Geometry: final body of the model. Coordinates: model frame, mm. Face numbers are marked on the shaded views. A direction names the side the tool comes from. Coordinates: 2 decimals unless noted, no trailing zeros. Write each loop counter-clockwise with the first axis right and the second up, starting at its lowest first coordinate (ties: lowest second). Pieces come first, ordered by that corner, then holes. Notation, with made-up numbers: M 74,-21.5 L 126,-21.5 A10 ccw 126,-4.5 Z; hole C 24,20.5 d8. An arc over 180 degrees is marked long. Write item = value, one per line. Start each with the question number.
Item 1: Reachability of the marked faces 1, 2 and 3 from +Z, -Z, +X, -X, +Y, -Y: full face, straight path, thin tool, end or side. Return the list, or none.
Item 2: Ray query, L1, parallel to X at y = 2.8, z = 0; L2, parallel to X at y = 0.7, z = 0; L3, parallel to Z at x = -14.5, y = 2.5. Return the intervals inside material, ascending. Write a range as [from, to].
Item 3: Section D-D on x = 16.5. Output: boundary loops of the cut face in (y, z).
Item 4: First-contact query: pin 1 Ø10 at (x, z) = (-3.5, -15) entering from -Y; pin 2 Ø5 at (x, z) = (3, 0.5) entering from +Y; pin 3 Ø4 at (x, z) = (13.5, 0) entering from +Y; pin 4 Ø4 at (y, z) = (2, 6.5) entering from -X. Flat tips, straight axial feed; report the tip coordinate or a pass-through.
Item 5: Section A-A on x = -14. Output: boundary loops of the cut face in (y, z).
Item 6: Section C-C on x = 12.5. Output: boundary loops of the cut face in (y, z), plus the area to 3 significant figures.
from build123d import *

# Parameters (mm, degrees)
SKETCH_1_R          = 20
EXTRUDE_1_DEPTH     = 3.2
SKETCH_2_R          = 5
EXTRUDE_2_DEPTH     = 6
SKETCH_3_R          = 11.669468733
SKETCH_3_R_2        = 9.545408708
CUT_EXTRUDE_1_DEPTH = 1
SKETCH_4_R          = 1.425
EXTRUDE_3_DEPTH     = 4
SKETCH_5_R          = 17.435273898
SKETCH_5_R_2        = 15.634190673
CUT_EXTRUDE_2_DEPTH = 1
SKETCH_6_R          = 10.034081131
SKETCH_6_R_2        = 8.408881881
CUT_EXTRUDE_3_DEPTH = 1


with BuildPart() as part:
    # 草图1 → 凸台-拉伸1 (new body)
    with BuildSketch(Plane(origin=(0, 0, 0), x_dir=(1, 0, 0), z_dir=(0, 1, 0))):
        with Locations(Location((0, 0, 0), (0, 0, 270))):
            Circle(SKETCH_1_R)
    extrude(amount=EXTRUDE_1_DEPTH)

    # 草图2 → 凸台-拉伸2 (add)
    with BuildSketch(Plane.XZ):
        with Locations(Location((0, 0, 0), (0, 0, 270))):
            Circle(SKETCH_2_R)
    extrude(amount=EXTRUDE_2_DEPTH)

    # 草图3 → 切除-拉伸1 (cut)
    with BuildSketch(Plane.XZ):
        with Locations(Location((0, 0, 0), (0, 0, 270))):
            Circle(SKETCH_3_R)
        with Locations(Location((0, 0, 0), (0, 0, 270))):
            Circle(SKETCH_3_R_2, mode=Mode.SUBTRACT)
    extrude(amount=-CUT_EXTRUDE_1_DEPTH, mode=Mode.SUBTRACT)

    # 草图4 → 凸台-拉伸3 (add)
    with BuildSketch(Plane(origin=(0, 3.2, 0), x_dir=(1, 0, 0), z_dir=(0, 1, 0))):
        with Locations(Location((0, 0, 0), (0, 0, 270))):
            Circle(SKETCH_4_R)
    extrude(amount=EXTRUDE_3_DEPTH)

    # 草图5 → 切除-拉伸2 (cut)
    with BuildSketch(Plane(origin=(0, 3.2, 0), x_dir=(1, 0, 0), z_dir=(0, 1, 0))):
        with Locations(Location((0, 0, 0), (0, 0, 270))):
            Circle(SKETCH_5_R)
        with Locations(Location((0, 0, 0), (0, 0, 270))):
            Circle(SKETCH_5_R_2, mode=Mode.SUBTRACT)
    extrude(amount=-CUT_EXTRUDE_2_DEPTH, mode=Mode.SUBTRACT)

    # 草图6 → 切除-拉伸3 (cut)
    with BuildSketch(Plane(origin=(0, 3.2, 0), x_dir=(1, 0, 0), z_dir=(0, 1, 0))):
        with Locations(Location((0, 0, 0), (0, 0, 270))):
            Circle(SKETCH_6_R)
        with Locations(Location((0, 0, 0), (0, 0, 270))):
            Circle(SKETCH_6_R_2, mode=Mode.SUBTRACT)
    extrude(amount=-CUT_EXTRUDE_3_DEPTH, mode=Mode.SUBTRACT)


solid = part.part
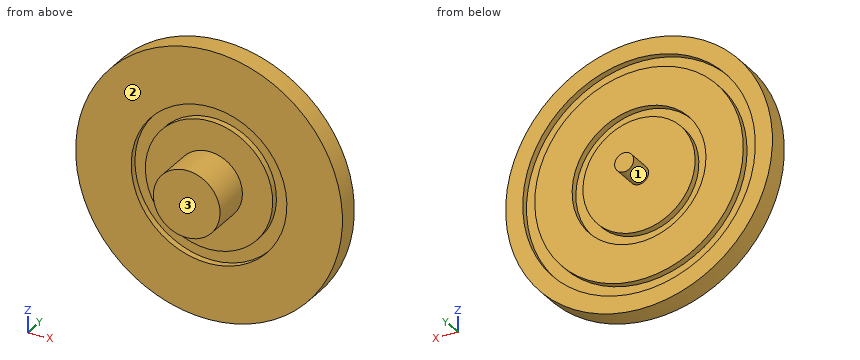
Responses:
q1.face_1 = +Y
q1.face_2 = -Y
q1.face_3 = +Z, -Z, +X, -X, -Y
q2.L1 = [-20, -17.44], [-15.63, -10.03], [-8.41, 8.41], [10.03, 15.63], [17.44, 20]
q2.L2 = [-20, -11.67], [-9.55, 9.55], [11.67, 20]
q2.L3 = [-13.77, -9.68], [-5.85, 5.85], [9.68, 13.77]
q3.outline = M 0,-11.3 L 3.2,-11.3 L 3.2,-5.63 L 2.2,-5.63 L 2.2,5.63 L 3.2,5.63 L 3.2,11.3 L 0,11.3 Z
q4.pin_1 = 0
q4.pin_2 = 7.2
q4.pin_3 = 3.2
q4.pin_4 = -19.49
q5.outline = M 0,-14.28 L 3.2,-14.28 L 3.2,-10.39 L 2.2,-10.39 L 2.2,-6.96 L 3.2,-6.96 L 3.2,6.96 L 2.2,6.96 L 2.2,10.39 L 3.2,10.39 L 3.2,14.28 L 0,14.28 Z
q6.outline = M 0,-15.61 L 3.2,-15.61 L 3.2,-12.15 L 2.2,-12.15 L 2.2,-9.39 L 3.2,-9.39 L 3.2,9.39 L 2.2,9.39 L 2.2,12.15 L 3.2,12.15 L 3.2,15.61 L 0,15.61 Z
q6.area = 94.4 mm²
